```python
from build123d import *

# Parameters (mm, degrees)
BOSS_EXTRUDE1_DEPTH = 20


with BuildPart() as part:
    # Sketch1 → Boss-Extrude1 (new body)
    with BuildSketch(Plane.XY):
        with BuildLine():
            Line((0, 0), (0, 1500))
            Line((0, 1500), (1800, 1500))
            Line((1800, 1500), (1800, 950))
            Line((1800, 950), (850, 950))
            ThreePointArc((850, 950), (637.867965644, 862.132034356), (550, 650))
            Line((550, 650), (550, 0))
            Line((550, 0), (0, 0))
        make_face()
    extrude(amount=BOSS_EXTRUDE1_DEPTH)


solid = part.part
```
Check sheet for the modelled part. Datum: model origin and axes. Units: mm. Round coordinates to 2 decimals unless told otherwise and drop trailing zeros. Write each loop counter-clockwise with the first axis right and the second up, starting at its lowest first coordinate (ties: lowest second). Pieces come first, ordered by that corner, then holes. Notation, with made-up numbers: M 66.5,38.25 L 120.5,38.25 A24 ccw 120.5,50.25 Z; hole C 25,44.25 d7. An arc over 180 degrees is marked long. Write item = value, one per line. Start each with the question number.
1. Section check A-A, the plane z = 16.25. Record the cut outline in (x, y), then the cut area to 3 significant figures.
2. Gauge pin test, flat ends, axial feed: pin 1 (4 mm diameter, centred on y = 1025.5, z = 7.5, fed in from -X); pin 2 (6 mm diameter, centred on x = 1276.5, z = 9, fed in from -Y). Record the tip position at first contact, or that the pin passes through.
3. Section check B-B, the plane x = 1253.5. Record the cut outline in (y, z).
4. Scan lines: line 1 (X direction, y = 665, z = 12); line 2 (X direction, y = 278, z = 15.5); line 3 (Y direction, x = 1300, z = 7.5). Record each from-to range of solid material in increasing order. Write a range as [from, to].
5. Section check C-C, the plane y = 237. Record the cut outline in (x, z).
Results found:
q1.outline = M 0,0 L 550,0 L 550,650 A300 cw 850,950 L 1800,950 L 1800,1500 L 0,1500 Z
q1.area = 1,530,000 mm^2
q2.pin_1 = 0
q2.pin_2 = 950
q3.outline = M 950,0 L 1500,0 L 1500,20 L 950,20 Z
q4.line_1 = [0, 550.38]
q4.line_2 = [0, 550]
q4.line_3 = [950, 1500]
q5.outline = M 0,0 L 550,0 L 550,20 L 0,20 Z
